```python
from build123d import *

# Parameters (mm, degrees)
SKETCH_1_W          = 570
SKETCH_1_H          = 535
EXTRUDE_1_DEPTH     = 5
FILLET_1_R          = 10
SKETCH_4_W          = 260
SKETCH_4_H          = 20
SKETCH_4_W_2        = 20
SKETCH_4_H_2        = 260
EXTRUDE_2_DEPTH     = 5
SKETCH_5_R          = 2.2
CUT_EXTRUDE_2_DEPTH = 420.17329352
FILLET_2_R          = 5


with BuildPart() as part:
    # 草图1 → 凸台-拉伸1 (new body)
    with BuildSketch(Plane.XY):
        Rectangle(SKETCH_1_W, SKETCH_1_H)
    extrude(amount=EXTRUDE_1_DEPTH)

    # 圆角1
    fillet_1_edges = [part.edges().sort_by_distance(p)[0] for p in [
        (285, -267.5, 2.5),
        (-285, -267.5, 2.5),
        (-285, 267.5, 2.5),
        (285, 267.5, 2.5),
    ]]
    fillet(fillet_1_edges, radius=FILLET_1_R)

    # 草图4 → 凸台-拉伸2 (add)
    with BuildSketch(Plane(origin=(0, 0, 0), x_dir=(-1, 0, 0), z_dir=(0, 0, -1))):
        with Locations((0, 277.5)):
            Rectangle(SKETCH_4_W, SKETCH_4_H)
        with Locations((295, 0)):
            Rectangle(SKETCH_4_W_2, SKETCH_4_H_2)
        with Locations((0, -277.5)):
            Rectangle(SKETCH_4_W, SKETCH_4_H)
        with Locations((-295, 0)):
            Rectangle(SKETCH_4_W_2, SKETCH_4_H_2)
    extrude(amount=-EXTRUDE_2_DEPTH)

    # 草图5 → 切除-拉伸2 (cut, through all)
    with BuildSketch(Plane(origin=(0, 0, 0), x_dir=(-1, 0, 0), z_dir=(0, 0, -1))):
        with Locations((-100, 280)):
            Circle(SKETCH_5_R)
        with Locations(Location((100, 280, 0), (0, 0, 180))):
            Circle(SKETCH_5_R)
        with Locations((290, 100)):
            Circle(SKETCH_5_R)
        with Locations(Location((290, -100, 0), (0, 0, 180))):
            Circle(SKETCH_5_R)
        with Locations((100, -280)):
            Circle(SKETCH_5_R)
        with Locations(Location((-100, -280, 0), (0, 0, 180))):
            Circle(SKETCH_5_R)
        with Locations((-290, -100)):
            Circle(SKETCH_5_R)
        with Locations(Location((-290, 100, 0), (0, 0, 180))):
            Circle(SKETCH_5_R)
    extrude(amount=-CUT_EXTRUDE_2_DEPTH, mode=Mode.SUBTRACT)

    # 圆角2
    fillet_2_edges = [part.edges().sort_by_distance(p)[0] for p in [
        (130, 287.5, 2.5),
        (130, 267.5, 2.5),
        (-130, 267.5, 2.5),
        (-130, 287.5, 2.5),
        (-305, -130, 2.5),
        (-305, 130, 2.5),
        (-285, 130, 2.5),
        (-285, -130, 2.5),
        (-130, -287.5, 2.5),
        (-130, -267.5, 2.5),
        (130, -267.5, 2.5),
        (130, -287.5, 2.5),
        (285, -130, 2.5),
        (285, 130, 2.5),
        (305, 130, 2.5),
        (305, -130, 2.5),
    ]]
    fillet(fillet_2_edges, radius=FILLET_2_R)


solid = part.part
```
Check sheet for the modelled part. Datum: model origin and axes. Units: mm. Give positions to 0.01 mm unless a question says otherwise; leave off trailing zeros. Write each loop counter-clockwise with the first axis right and the second up, starting at its lowest first coordinate (ties: lowest second). Pieces come first, ordered by that corner, then holes.
Item 1: Scan lines: L1, parallel to Y at x = -100, z = 1.7; L2, parallel to Y at x = 99.5, z = 3.9; L3, parallel to X at y = -280, z = 3.45. Record each from-to range of solid material in increasing order.
Item 2: Cross-section at B-B (z = 1.95). Count the separate pieces of the cut face and the enclosed holes in it, and give its area (3 significant figures).
Item 3: Gauge pin test, flat ends, axial feed: pin 1 (2 mm diameter, centred on x = -186.5, z = 2.5, fed in from +Y); pin 2 (2 mm diameter, centred on y = -153, z = 4, fed in from -X); pin 3 (1.5 mm diameter, centred on y = 277, z = 3, fed in from -X); pin 4 (2.5 mm diameter, centred on x = -100, y = 280, fed in from +Z). Record the tip position at first contact, or that the pin passes through.
Item 4: Cross-section at A-A (x = -148.5). Enter the section's corners in (y, z).
Item 5: Cross-section at C-C (y = 176). Enter the section's corners in (x, z).
Report:
1. L1: y = -287.5 to -282.2, -277.8 to 277.8, 282.2 to 287.5
1. L2: y = -287.5 to -282.14, -277.86 to 277.86, 282.14 to 287.5
1. L3: x = -130 to -102.2, -97.8 to 97.8, 102.2 to 130
2. separate pieces: 1
2. enclosed holes: 8
2. area: 326,000 mm2
3. pin 1: stops at y = 267.5
3. pin 2: stops at x = -285
3. pin 3: stops at x = -130
3. pin 4: passes through
4. outline: (-267.5, 0) - (267.5, 0) - (267.5, 5) - (-267.5, 5) - close
5. outline: (-285, 0) - (285, 0) - (285, 5) - (-285, 5) - close
